from build123d import *

# Parameters (mm, degrees)
EXTRUDE_1_DEPTH     = 15
CUT_EXTRUDE_1_DEPTH = 20
MM_1_D              = 6
HOLE_WIZARD_M6_1_D  = 5


with BuildPart() as part:
    # 草图1 → 凸台-拉伸1 (new body)
    with BuildSketch(Plane.XY):
        with BuildLine():
            Line((-145.547396155, 197.773537563), (-142.072104357, 202.664585193))
            Line((-142.072104357, 202.664585193), (-71.595844229, 152.588285115))
            ThreePointArc((-71.595844229, 152.588285115), (-70.97220164, 152.200308518), (-70.305827411, 151.891437501))
            Line((-70.305827411, 151.891437501), (20.980591756, 116.19178332))
            Line((20.980591756, 116.19178332), (18.795316776, 110.603888076))
            Line((18.795316776, 110.603888076), (-73.179003731, 146.5725619))
            ThreePointArc((-73.179003731, 146.5725619), (-73.84537796, 146.881432918), (-74.469020549, 147.269409515))
            Line((-74.469020549, 147.269409515), (-145.547396155, 197.773537563))
        make_face()
    extrude(amount=EXTRUDE_1_DEPTH)

    # 草图3 → 切除-拉伸1 (cut)
    with BuildSketch(Plane(origin=(48.026613519, 67.591577297, 0), x_dir=(0.8151746049568696, -0.5792152997231786, 0), z_dir=(0.5792152997231786, 0.8151746049568696, 0))):
        Polygon((-233.2, -7.5), (-146.744583334, -15), (-233.2, -15), align=None)
    extrude(amount=-CUT_EXTRUDE_1_DEPTH, mode=Mode.SUBTRACT)

    # 大小mm 暗销孔1 (through all)
    with Locations(Plane(origin=(48.026613519, 67.591577297, 0), x_dir=(0.8151746049568697, -0.5792152997231785, 0), z_dir=(0.5792152997231785, 0.8151746049568697, 0))):
        with Locations((-200.523492287, -4.870838518), (-171.040138216, -4.870838518)):
            Hole(MM_1_D / 2)

    # M6 螺纹孔1 (through all)
    with Locations(Plane(origin=(48.026613519, 67.591577297, 0), x_dir=(0.8151746049568697, -0.5792152997231785, 0), z_dir=(0.5792152997231785, 0.8151746049568697, 0))):
        with Locations((-190.523492287, -4.870838518), (-181.040138216, -4.870838518)):
            Hole(HOLE_WIZARD_M6_1_D / 2)


solid = part.part
Design review of the part built by this model. Coordinates are the model's own, in mm. Give positions to 0.01 mm unless a question says otherwise; leave off trailing zeros. Loops run counter-clockwise (first coordinate to the right, second up) from the corner with the lowest first, then second, coordinate; pieces in that order, holes last. Notation, with made-up numbers: (30, 47) - (44, 47) arc R24 ccw to (44, 84) - close; hole circle Ø8 at (-6.75, 88). An arc over 180 degrees is marked (long way). Write item = value, one per line.
1) Clearance check with flat-ended pins moving along their axes: pin 1 Ø3 at (x, z) = (-122.5, 7) entering from -Y; pin 2 Ø6 at (x, z) = (-87.5, 10) entering from -Y; pin 3 Ø1 at (x, z) = (-65, 8.5) entering from -Y. State where each tip first meets the part, or that it passes through.
Result sheet:
pin_1 = 180.33
pin_2 = 154.4
pin_3 = 143.18
2) Take a section at B-B on y = 154.5. State the section outline as (x, z) points, and give its area (3 significant figures).
Result sheet:
outline = (-84.65, 0) - (-74.29, 0) - (-74.29, 14.71) - (-84.65, 13.98) - close
area = 149 mm2
3) To check wall thickness, follow line 1 (Y direction, x = -38.5, z = 1); line 2 (X direction, y = 162, z = 5); line 3 (Y direction, x = -54, z = 11.75). State the ranges of each line that lie inside material, in increasing order.
Result sheet:
line_1 = 133.01 to 139.45
line_2 = -91.04 to -84.84
line_3 = 139.07 to 145.51
4) Draft analysis for pull direction Y (two halves, no side actions). For faces 1 (the face through (-143.834, 200.185, 3.698)), 2 (the face through (-103.197, 171.311, 5.828)), 3 (the face through (-109.511, 172.168, 7.395)), state which applies: +Y half, -Y half, draft (parallel to the pull), parting line (faces both ways), or undercut.
Result sheet:
face_1 = +Y half
face_2 = undercut
face_3 = -Y half
5) Take a section at A-A on z = 12. State the section outline as (x, y) points.
Result sheet:
outline = (-103.26, 167.73) - (-74.47, 147.27) arc R6 ccw to (-73.18, 146.57) - (18.8, 110.6) - (20.98, 116.19) - (-70.31, 151.89) arc R6 cw to (-71.6, 152.59) - (-99.79, 172.62) - close
6) Take a section at C-C on x = -130. State the section outline as (y, z) points.
Result sheet:
outline = (186.73, 0) - (194.09, 0) - (194.09, 8.78) - (186.73, 9.15) - close
